from build123d import *

# Parameters (mm, degrees)
SKETCH1_W                                            = 22
SKETCH1_H                                            = 14.5
BOSS_EXTRUDE1_DEPTH                                  = 7.3
SKETCH2_R                                            = 4.75
CUT_EXTRUDE1_DEPTH                                   = 16.061623418
F_3_4_3_4_DIAMETER_HOLE1_D                           = 3.4
SKETCH5_W                                            = 15
SKETCH5_H                                            = 1
CUT_EXTRUDE2_DEPTH                                   = 16.061623418
SKETCH6_W                                            = 1
SKETCH6_H                                            = 6.75
CUT_EXTRUDE3_DEPTH                                   = 17
FILLET1_R                                            = 2
FILLET2_R                                            = 1
SKETCH7_W                                            = 1.25
SKETCH7_H                                            = 6.75
HOLE_SIZE_PER_SOCKET_HEAD_CAP_SCREW_TYPE_D           = 3.4
HOLE_SIZE_PER_SOCKET_HEAD_CAP_SCREW_TYPE_DEPTH       = 7.749
HOLE_SIZE_PER_SOCKET_HEAD_CAP_SCREW_TYPE_CBORE_D     = 6
HOLE_SIZE_PER_SOCKET_HEAD_CAP_SCREW_TYPE_CBORE_DEPTH = 3.4
CUT_EXTRUDE4_DEPTH                                   = 3.4
CHAMFER1_SIZE                                        = 1


with BuildPart() as part:
    # Sketch1 → Boss-Extrude1 (new body)
    with BuildSketch(Plane.XY):
        Rectangle(SKETCH1_W, SKETCH1_H)
    extrude(amount=BOSS_EXTRUDE1_DEPTH)

    # Sketch2 → Cut-Extrude1 (cut, through all)
    with BuildSketch(Plane.XY.offset(7.3)):
        with Locations((4, -0.75)):
            Circle(SKETCH2_R)
    extrude(amount=-CUT_EXTRUDE1_DEPTH, mode=Mode.SUBTRACT)

    # Ø3.4 (3.4) Diameter Hole1 (through all)
    with Locations(Plane.XY.offset(7.3)):
        with Locations((-8, -3.75)):
            Hole(F_3_4_3_4_DIAMETER_HOLE1_D / 2)

    # Sketch5 → Cut-Extrude2 (cut, through all)
    with BuildSketch(Plane.XY.offset(7.3)):
        Rectangle(SKETCH5_W, SKETCH5_H)
    extrude(amount=-CUT_EXTRUDE2_DEPTH, mode=Mode.SUBTRACT)

    # Sketch6 → Cut-Extrude3 (cut)
    with BuildSketch(Plane.XY.offset(7.3)):
        with Locations((-7, 3.875)):
            Rectangle(SKETCH6_W, SKETCH6_H)
    extrude(amount=-CUT_EXTRUDE3_DEPTH, mode=Mode.SUBTRACT)

    # Fillet1
    fillet1_edges = [part.edges().sort_by_distance(p)[0] for p in [
        (-7.5, -0.5, 3.65),
    ]]
    fillet(fillet1_edges, radius=FILLET1_R)

    # Fillet2
    fillet2_edges = [part.edges().sort_by_distance(p)[0] for p in [
        (-6.5, 0.5, 3.65),
    ]]
    fillet(fillet2_edges, radius=FILLET2_R)

    # Sketch7 → M3 Tapped Hole1 (revolve, cut)
    with BuildSketch(Plane(origin=(-3, -0.5, 3.65), x_dir=(0, 0, 1), z_dir=(1, 0, 0))):
        with Locations((0.625, 3.375)):
            Rectangle(SKETCH7_W, SKETCH7_H)
    revolve(axis=Axis((-3, 5.85, 3.65), (0, -1, 0)), mode=Mode.SUBTRACT)

    # Hole size per socket head cap screw type 3
    with Locations(Plane(origin=(0, 7.25, 0), x_dir=(1, 0, 0), z_dir=(0, 1, 0))):
        with Locations((-3, -3.65)):
            CounterBoreHole(HOLE_SIZE_PER_SOCKET_HEAD_CAP_SCREW_TYPE_D / 2, HOLE_SIZE_PER_SOCKET_HEAD_CAP_SCREW_TYPE_CBORE_D / 2, HOLE_SIZE_PER_SOCKET_HEAD_CAP_SCREW_TYPE_CBORE_DEPTH, depth=HOLE_SIZE_PER_SOCKET_HEAD_CAP_SCREW_TYPE_DEPTH)

    # Sketch13 → Cut-Extrude4 (cut)
    with BuildSketch(Plane.XY.offset(7.3)):
        with BuildLine():
            Line((-8, -6.6), (-13.475777531, -6.6))
            ThreePointArc((-13.475777531, -6.6), (-16.325777531, -3.75), (-13.475777531, -0.9))
            Line((-13.475777531, -0.9), (-8, -0.9))
            ThreePointArc((-8, -0.9), (-5.15, -3.75), (-8, -6.6))
        make_face()
    extrude(amount=-CUT_EXTRUDE4_DEPTH, mode=Mode.SUBTRACT)

    # Chamfer1
    chamfer1_edges = [part.edges().sort_by_distance(p)[0] for p in [
        (11, -7.25, 3.65),
        (-11, 7.25, 3.65),
        (11, 7.25, 3.65),
    ]]
    chamfer(chamfer1_edges, length=CHAMFER1_SIZE)


solid = part.part
Could you check a few things on this model? Use its own coordinates, in mm. A direction names the side the tool comes from. Give positions to 0.01 mm unless a question says otherwise; leave off trailing zeros. Order: outer loops, then holes, each group sorted by start corner. A loop starts at its lowest first (then second) coordinate and runs counter-clockwise, first axis right, second up. Notation, with made-up numbers: (-2.5, 85) -> (30.5, 85) arc R36 ccw to (30.5, 121) -> close; hole circle Ø8 at (67, 78). An arc over 180 degrees is marked (long way). Answer in a Markdown table with one row per item. Add a question column.
Item 1: We'd pull the mould along X, two halves only. Please class faces 1 (the flat face through (-11, 1, 3)), 2 (the flat face through (-7.5, 4, 4)), 3 (the flat face through (3, 7.25, 4)), 4 (the flat face through (10.49, -6.76, 3.6)): pulls with the +X half, pulls with the -X half, needs draft (parallel to the pull), parting line crosses it, or undercut.
Item 2: Imagine slicing it at C-C (y = -1.25). List the corners of the cut face in (x, z) for me, and give its area (3 significant figures).
Item 3: Imagine slicing it at B-B (x = -3). List the corners of the cut face in (y, z) for me.
Item 4: For faces 5 (the flat face through (-10.49, 6.76, 3.6)), 6 (the cylindrical face through (-6.199, 0.785, 3.599)), 7 (the flat face through (-3, 3.85, 6)), 8 (the flat face through (-9, -6.6, 6)), which set-ups out of +Z, -Z, +X, -X, +Y, -Y let a thin tool reach every point of the face, with its end or its side?
Item 5: Imagine slicing it at A-A (y = 2.75). List the corners of the cut face in (x, z) for me, and give its area (3 significant figures).
Item 6: Please list where these lines run through material, in increasing order: probe 1 along Y at (x, z) = (-5, 7); probe 2 along Y at (x, z) = (-8, 5.5); probe 3 along X at (y, z) = (5.5, 4).
Item 7: I'm going to push flat-ended pins straight in: P1, Ø3, axis at x = 1, y = -0.5, coming from the +Z side; P2, Ø1.7, axis at x = -8, y = -5, coming from the +Z side; P3, Ø4, axis at x = -3, z = 3.65, coming from the +Y side. Where does each tip first touch, or does it pass through?
Item 8: Imagine slicing it at D-D (z = 4.5). Count the separate pieces of the cut face and the enclosed holes in it, and give its area (3 significant figures).
Result:
| question | item | result |
|---|---|---|
| 1 | face 1 | pulls with the -X half |
| 1 | face 2 | undercut |
| 1 | face 3 | needs draft |
| 1 | face 4 | pulls with the +X half |
| 2 | outline | (-11, 0) -> (-0.72, 0) -> (-0.72, 7.3) -> (-6.63, 7.3) -> (-6.63, 3.9) -> (-11, 3.9) -> close; (8.72, 0) -> (11, 0) -> (11, 7.3) -> (8.72, 7.3) -> close; hole circle Ø2.5 at (-3, 3.65) |
| 2 | area | 71.9 mm2 |
| 3 | outline | (-7.25, 0) -> (-0.5, 0) -> (-0.5, 2.4) -> (-7.25, 2.4) -> close; (-7.25, 4.9) -> (-0.5, 4.9) -> (-0.5, 7.3) -> (-7.25, 7.3) -> close; (0.5, 0) -> (7.25, 0) -> (7.25, 0.65) -> (3.85, 0.65) -> (3.85, 1.95) -> (0.5, 1.95) -> close; (0.5, 5.35) -> (3.85, 5.35) -> (3.85, 6.65) -> (7.25, 6.65) -> (7.25, 7.3) -> (0.5, 7.3) -> close |
| 4 | face 5 | +Z, -Z, -X, +Y |
| 4 | face 6 | +Z, -Z |
| 4 | face 7 | +Y |
| 4 | face 8 | +Z, -X |
| 5 | outline | (-11, 0) -> (-7.5, 0) -> (-7.5, 7.3) -> (-11, 7.3) -> close; (-6.5, 0) -> (0.79, 0) -> (0.79, 7.3) -> (-6.5, 7.3) -> close; (7.21, 0) -> (11, 0) -> (11, 7.3) -> (7.21, 7.3) -> close; hole circle Ø3.4 at (-3, 3.65) |
| 5 | area | 97.3 mm2 |
| 6 | probe 1 | -7.25 to -0.5, 0.5 to 7.25 |
| 6 | probe 2 | -7.25 to -6.6, -0.9 to 7.25 |
| 6 | probe 3 | -11 to -7.5, -6.5 to -5.98, -0.02 to 11 |
| 7 | P1 | through |
| 7 | P2 | z = 3.9 |
| 7 | P3 | y = 3.85 |
| 8 | separate pieces | 3 |
| 8 | enclosed holes | 0 |
| 8 | area | 162 mm2 |
